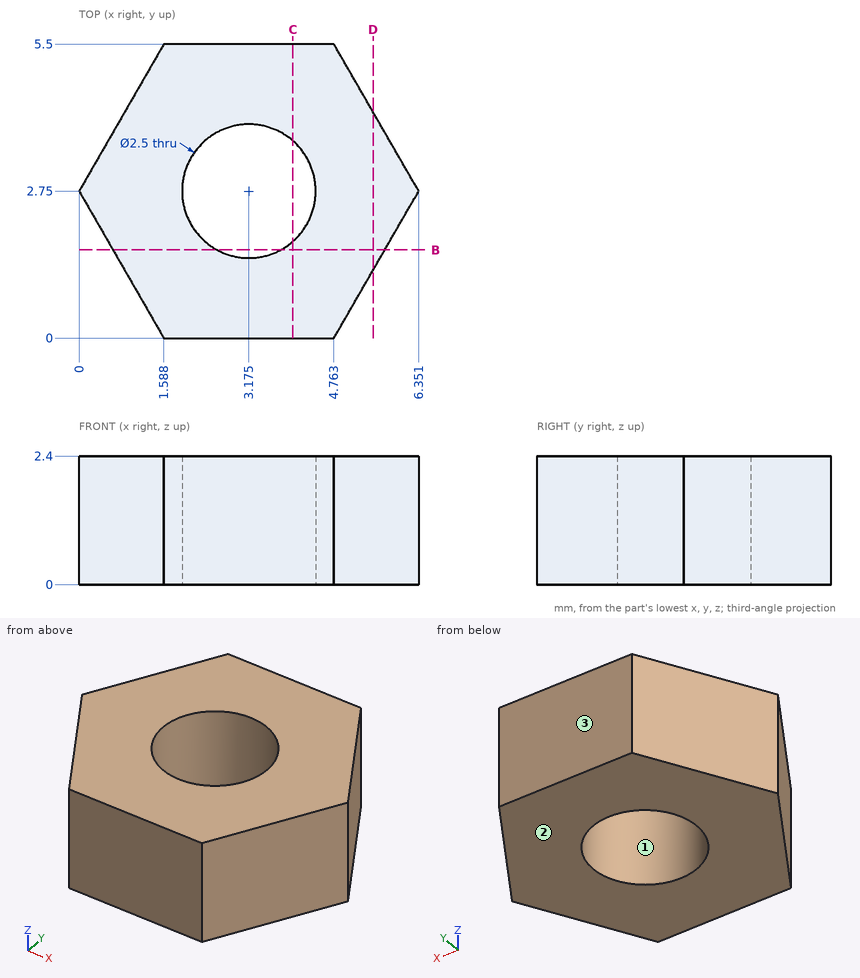
Job drawing, mm, ordinate dimensions from the low corner. One solid piece. Give positions to 0.01 mm unless a question says otherwise; leave off trailing zeros. Loops run counter-clockwise (first coordinate to the right, second up) from the corner with the lowest first, then second, coordinate; pieces in that order, holes last. Notation, with made-up numbers: (66.25, 47.25) - (120.25, 47.25) arc R25 ccw to (120.25, 60.25) - close; hole circle Ø3 at (-17.5, 69.25). An arc over 180 degrees is marked (long way). Use one line per item in the form item = value.
(1) Cut at D-D (x = 5.5). Give the cut face in (y, z).
Determined:
outline = (1.28, 0) - (4.22, 0) - (4.22, 2.4) - (1.28, 2.4) - close
(2) Pull direction Y, two halves, no side cores. Call the marked faces 1, 2 and 3: pulls with the +Y half, pulls with the -Y half, needs draft (parallel to the pull), parting line crosses it, or undercut.
Determined:
face_1 = undercut
face_2 = needs draft
face_3 = pulls with the +Y half
(3) Drill centre lines: L1, parallel to Y at x = 4, z = 2.15; L2, parallel to X at y = 3.05, z = 0.15 (1 decimal); L3, parallel to Y at x = 3, z = 0.45. Where is each one in solid material? Low to high.
Determined:
L1 = 0 to 1.81, 3.69 to 5.5
L2 = 0.2 to 2, 4.4 to 6.2
L3 = 0 to 1.51, 3.99 to 5.5
(4) Drop a flat-ended pin along its axis: P1, Ø1, axis at x = 5.5, z = 0.5, coming from the -Y side. Give the stop position or say it passes through.
Determined:
P1 = 0.41
(5) Cut at C-C (x = 4). Give the cut face in (y, z).
Determined:
outline = (0, 0) - (1.81, 0) - (1.81, 2.4) - (0, 2.4) - close; (3.69, 0) - (5.5, 0) - (5.5, 2.4) - (3.69, 2.4) - close
(6) Cut at B-B (y = 1.65). Give the cut face in (x, z) (1 decimal).
Determined:
outline = (0.6, 0) - (2.6, 0) - (2.6, 2.4) - (0.6, 2.4) - close; (3.8, 0) - (5.7, 0) - (5.7, 2.4) - (3.8, 2.4) - close
